Read the model definition and answer for the solid it produces. Units are mm, in the model's axes. A direction names the side the tool comes from. Give positions to 0.01 mm unless a question says otherwise; leave off trailing zeros. Loops run counter-clockwise (first coordinate to the right, second up) from the corner with the lowest first, then second, coordinate; pieces in that order, holes last. Notation, with made-up numbers: (-30, 5.5) - (16, 5.5) arc R16 cw to (16, 14.5) - close; hole circle Ø8 at (43, -2). An arc over 180 degrees is marked (long way). Put each result on its own line as item: value. Start each with the question number.
1. For a pull along Z with two mould halves and no side action, classify faces 1 (the cylindrical face through (-7.65, -28.38, -0.07)), 2 (the flat face through (0, -33.5, 0)), 3 (the flat face through (0, 0, 4)), 4 (the flat face through (0, 0, -4)) as released by +Z, released by -Z, zero draft, split by the parting line, or undercut.
2. A cutting plane is placed at A-A, the plane y = 30. Determine the outline of the cut face in (x, z), plus the area to 3 significant figures.
3. Consider L1, parallel to Z at x = 6, y = -27.5; L2, parallel to Y at x = -8, z = 1; L3, parallel to Y at x = -5.5, z = 1. Determine where each line is inside the solid, lowest interval first. Write a range as from..to.
4. A cutting plane is placed at B-B, the plane y = -24.5. Determine the outline of the cut face in (x, z).
5. Given pin 1 Ø2 at (x, y) = (-8, 30) entering from +Z; pin 2 Ø4 at (x, z) = (6, 0) entering from -Y, each flat-ended and moving along its own axis, determine where each tip first touches the part or whether it passes through.
6. For faces 5 (the flat face through (0, 33.5, 0)), 6 (the cylindrical face through (4.35, -28.38, -0.07)), determine the directions among +Z, -Z, +X, -X, +Y, -Y from which every point of the face is accessible in a straight line to the end or side of a thin tool.
```python
from build123d import *

# Parameters (mm, degrees)
SKETCH_1_W             = 20
SKETCH_1_H             = 67
EXTRUDE_1_DEPTH        = 4
HOLE_WIZARD_M3_1_D     = 2.5
HOLE_WIZARD_M4_1_D     = 3.3
HOLE_WIZARD_M4_1_DEPTH = 10.1
HOLE_WIZARD_M4_1_TIP   = 0.991420021
CHAMFER_1_SIZE         = 1


with BuildPart() as part:
    # 草图1 → 凸台-拉伸1 (new, symmetric)
    with BuildSketch(Plane.XY):
        Rectangle(SKETCH_1_W, SKETCH_1_H)
    extrude(amount=EXTRUDE_1_DEPTH, both=True)

    # M3 螺纹孔1 (through all)
    with Locations(Plane(origin=(0, 0, -4), x_dir=(-1, 0, 0), z_dir=(0, 0, -1))):
        with Locations((8, 30)):
            Hole(HOLE_WIZARD_M3_1_D / 2)

    # M4 螺纹孔1
    with Locations(Plane(origin=(0, -33.5, 0), x_dir=(-1, 0, 0), z_dir=(0, -1, 0))):
        with Locations((6, 0), (-6, 0)):
            Hole(HOLE_WIZARD_M4_1_D / 2, depth=HOLE_WIZARD_M4_1_DEPTH)
            with Locations((0, 0, -(HOLE_WIZARD_M4_1_DEPTH + HOLE_WIZARD_M4_1_TIP / 2))):  # 118° drill point
                Cone(0, HOLE_WIZARD_M4_1_D / 2, HOLE_WIZARD_M4_1_TIP, mode=Mode.SUBTRACT)

    # 倒角1
    chamfer_1_edges = [part.edges().sort_by_distance(p)[0] for p in [
        (10, -33.5, 0),
        (-10, -33.5, 0),
        (-10, 33.5, 0),
        (10, 33.5, 0),
    ]]
    chamfer(chamfer_1_edges, length=CHAMFER_1_SIZE)


solid = part.part
```
Return value:
1. face 1: undercut
1. face 2: zero draft
1. face 3: released by +Z
1. face 4: released by -Z
2. outline: (-10, -4) - (-9.25, -4) - (-9.25, 4) - (-10, 4) - close; (-6.75, -4) - (10, -4) - (10, 4) - (-6.75, 4) - close
2. area: 140 mm2
3. L1: z = -4..-1.65, 1.65..4
3. L2: y = -33.5..28.75, 31.25..33.5
3. L3: y = -23.08..33.5
4. outline: (-10, -4) - (10, -4) - (10, 4) - (-10, 4) - close; hole circle Ø3.3 at (-6, 0); hole circle Ø3.3 at (6, 0)
5. pin 1: passes through
5. pin 2: stops at y = -33.5
6. face 5: +Z, -Z, +X, -X, +Y
6. face 6: -Y
